from build123d import *

# Parameters (mm, degrees)
BOSS_EXTRUDE1_DEPTH = 185
BOSS_EXTRUDE2_DEPTH = 35
CUT_EXTRUDE1_START  = -110
CUT_EXTRUDE1_DEPTH  = 32
CUT_EXTRUDE2_START  = 70
CUT_EXTRUDE2_DEPTH  = 32
SKETCH6_W           = 76.501144457
SKETCH6_H           = 19
LPATTERN1_COUNT     = 2
LPATTERN1_PITCH     = 180


with BuildPart() as part:
    # Sketch1 → Boss-Extrude1 (new, symmetric)
    with BuildSketch(Plane(origin=(0, 0, 0), x_dir=(0, 0, -1), z_dir=(1, 0, 0))):
        Polygon((0, 0), (0, 110.794919243), (50, 97.397459622), (50, 13.397459622), align=None)
    extrude(amount=BOSS_EXTRUDE1_DEPTH, both=True)

    # Sketch2 → Boss-Extrude2 (add)
    with BuildSketch(Plane.ZY.offset(185)):
        Polygon((0, 0), (-50, 0), (-50, 13.397459622), align=None)
    extrude(amount=-BOSS_EXTRUDE2_DEPTH)

    # Sketch3 → Cut-Extrude1 (cut, symmetric)
    with BuildSketch(Plane(origin=(0, 0, 0), x_dir=(0, 0, -1), z_dir=(1, 0, 0)).offset(CUT_EXTRUDE1_START)):
        Polygon((16.51733163, 4.425805671), (42.003158605, 99.540206815), (0, 110.794919243), (0, 0), align=None)
    extrude(amount=CUT_EXTRUDE1_DEPTH, both=True, mode=Mode.SUBTRACT)

    # Sketch4 → Cut-Extrude2 (cut, symmetric)
    with BuildSketch(Plane(origin=(0, 0, 0), x_dir=(0, 0, -1), z_dir=(1, 0, 0)).offset(CUT_EXTRUDE2_START)):
        Polygon((16.51733163, 4.425805671), (42.003158605, 99.540206815), (0, 110.794919243), (0, 0), align=None)
    extrude(amount=CUT_EXTRUDE2_DEPTH, both=True, mode=Mode.SUBTRACT)

    # Sketch6 → Cut-Revolve1 (revolve, cut)
    with BuildSketch(Plane(origin=(0, 54.390611447, -19.79656359), x_dir=(0, 0.342020143325663, 0.9396926207859105), z_dir=(0, 0.9396926207859105, -0.342020143325663)), mode=Mode.PRIVATE) as cut_revolve1_sk:
        with Locations((-25.35224184, -100.5)):
            Rectangle(SKETCH6_W, SKETCH6_H)
    cut_revolve1 = revolve(cut_revolve1_sk.sketch.rotate(Axis((-110, 31.16565465, -83.606607958), (0, 0.342020143325663, 0.9396926207859105)), 270), axis=Axis((-110, 31.16565465, -83.606607958), (0, 0.342020143325663, 0.9396926207859105)), mode=Mode.SUBTRACT)

    # LPattern1: Cut-Revolve1 ×2
    with Locations(*[(i * LPATTERN1_PITCH, 0, 0) for i in range(1, LPATTERN1_COUNT)]):
        add(cut_revolve1, mode=Mode.SUBTRACT)


solid = part.part
Source: CAD feature listing. Evaluate the final solid. Frame: model axes, mm. A direction names the side the tool comes from. Round coordinates to 2 decimals unless told otherwise and drop trailing zeros. Write each loop counter-clockwise with the first axis right and the second up, starting at its lowest first coordinate (ties: lowest second). Pieces come first, ordered by that corner, then holes. Notation, with made-up numbers: (28, -25.5) - (86, -25.5) arc R21 ccw to (86, 2.5) - close; hole circle Ø11 at (-24.5, 79). An arc over 180 degrees is marked (long way). Use CSV: the item, a comma, the result in double quotes. Start each with the question number.
(1) Set-up query: faces 4 (the face through (-150, 4, -36)), 5 (the face through (-3, 59, -50)), 6 (the face through (-78, 56, -16)). Return all of +Z, -Z, +X, -X, +Y, -Y with unobstructed straight access to the full face (end or side cutting, diameter ignored); none if empty.
(2) Cut plane C-C, the plane x = -7.5. Return loops of the section in (y, z).
(3) Mould query, pull axis Y, two halves, no side actions, for faces 1 (the face through (-117.28, 31.11, -32.45)), 2 (the face through (-88.219, 51.317, -29.082)), 3 (the face through (-142, 56, -16)). Classes: pulls with the +Y half, pulls with the -Y half, needs draft (parallel to the pull), parting line crosses it, or undercut.
(4) First-contact query: pin 1 Ø10 at (x, z) = (-105, -12) entering from -Y; pin 2 Ø1.5 at (x, z) = (-67.5, -37.5) entering from -Y; pin 3 Ø4 at (x, z) = (77, -41) entering from +Y. Flat tips, straight axial feed; report the tip coordinate or a pass-through.
(5) Cut plane A-A, the plane z = -11.5. Return loops of the section in (x, y), and give its area (3 significant figures).
(6) Cut plane D-D, the plane z = -34.5. Give the number of separate pieces and of enclosed holes in the cut face, and give its area (3 significant figures).
(7) Cut plane B-B, the plane y = 84. Return loops of the section in (x, z).
(8) Material intervals for probe 1 along X at (y, z) = (36.5, -21.5); probe 2 along X at (y, z) = (37, -42); probe 3 along Z at (x, y) = (95, 48), sorted ascending. Write a range as [from, to].
Geometry says:
1,face 4,"-Z, +X, -Y"
1,face 5,"-Z, +X, -X, +Y, -Y"
1,face 6,"+Z, +Y"
2,outline,"(0, 0) - (13.4, -50) - (97.4, -50) - (110.79, 0) - close"
3,face 1,"undercut"
3,face 2,"pulls with the +Y half"
3,face 3,"needs draft"
4,pin 1,"y = 4.43"
4,pin 2,"y = 9.85"
4,pin 3,"y = 99.54"
5,outline,"(-185, 0) - (-150, 0) - (-150, 3.08) - (-142, 3.08) - (-142, 107.71) - (-185, 107.71) - close; (-78, 3.08) - (38, 3.08) - (38, 107.71) - (-78, 107.71) - close; (102, 3.08) - (185, 3.08) - (185, 107.71) - (102, 107.71) - close"
5,area,"25,400 mm²"
6,separate pieces,"1"
6,enclosed holes,"2"
6,area,"28,200 mm²"
7,outline,"(-185, -50) - (185, -50) - (185, 0) - (102, 0) - (102, -37.84) - (38, -37.84) - (38, 0) - (-78, 0) - (-78, -37.84) - (-142, -37.84) - (-142, 0) - (-185, 0) - close"
8,probe 1,"[-185, -142], [-78, 38], [102, 185]"
8,probe 2,"[-185, -126.87], [-93.13, 53.13], [86.87, 185]"
8,probe 3,"[-50, -28.19]"
